Verification items for the finished model (mm, model axes). Face numbers are marked on the shaded views. A direction names the side the tool comes from. Round coordinates to 2 decimals unless told otherwise and drop trailing zeros. Write each loop counter-clockwise with the first axis right and the second up, starting at its lowest first coordinate (ties: lowest second). Pieces come first, ordered by that corner, then holes.
from build123d import *

# Parameters (mm, degrees)
FORMED_BRACKET_BODY_DEPTH = 150
BOSS_TUBE_SKETCH_R        = 112.5
BOSS_TUBE_SKETCH_R_2      = 87.5
BOSS_TUBE_225X170_DEPTH   = 170
BASE_HOLE_75_REACH        = 541.805
BASE_HOLE_SKETCH_R        = 37.5


with BuildPart() as part:
    # Bracket Profile Sketch → Formed Bracket Body (new, symmetric)
    with BuildSketch(Plane.XY):
        with BuildLine():
            Line((-475, 0), (-237.5, 0))
            ThreePointArc((-237.5, 0), (-202.144660941, -14.644660941), (-187.5, -50))
            Line((-187.5, -50), (-187.5, -188))
            ThreePointArc((-187.5, -188), (-181.642135624, -202.142135624), (-167.5, -208))
            Line((-167.5, -208), (167.5, -208))
            ThreePointArc((167.5, -208), (181.642135624, -202.142135624), (187.5, -188))
            Line((187.5, -188), (187.5, -50))
            ThreePointArc((187.5, -50), (202.144660941, -14.644660941), (237.5, 0))
            Line((237.5, 0), (475, 0))
            Line((475, 0), (475, -30))
            Line((475, -30), (237.5, -30))
            ThreePointArc((237.5, -30), (223.357864376, -35.857864376), (217.5, -50))
            Line((217.5, -50), (217.5, -188))
            ThreePointArc((217.5, -188), (202.855339059, -223.355339059), (167.5, -238))
            Line((167.5, -238), (-167.5, -238))
            ThreePointArc((-167.5, -238), (-202.855339059, -223.355339059), (-217.5, -188))
            Line((-217.5, -188), (-217.5, -50))
            ThreePointArc((-217.5, -50), (-223.357864376, -35.857864376), (-237.5, -30))
            Line((-237.5, -30), (-475, -30))
            Line((-475, -30), (-475, 0))
        make_face()
    extrude(amount=FORMED_BRACKET_BODY_DEPTH, both=True)

    # Boss Tube Sketch → Boss Tube Ø225x170 (add)
    with BuildSketch(Plane(origin=(0, -208, 0), x_dir=(1, 0, 0), z_dir=(0, 1, 0))):
        with Locations(Location((0, 0, 0), (0, 0, 180))):
            Circle(BOSS_TUBE_SKETCH_R)
        with Locations(Location((0, 0, 0), (0, 0, 180))):
            Circle(BOSS_TUBE_SKETCH_R_2, mode=Mode.SUBTRACT)
    extrude(amount=BOSS_TUBE_225X170_DEPTH)

    # Base Hole Sketch → Base Hole Ø75 (cut, up to next)
    with BuildSketch(Plane(origin=(0, -208, 0), x_dir=(1, 0, 0), z_dir=(0, 1, 0)), mode=Mode.PRIVATE) as base_hole_75_sk1:
        with Locations(Location((0, 0, 0), (0, 0, 180))):
            Circle(BASE_HOLE_SKETCH_R)
    base_hole_75_tool1 = extrude(base_hole_75_sk1.sketch, amount=-BASE_HOLE_75_REACH, mode=Mode.PRIVATE) & part.part
    add(base_hole_75_tool1.solids().sort_by_distance((0, -208, 0))[0], mode=Mode.SUBTRACT)


solid = part.part
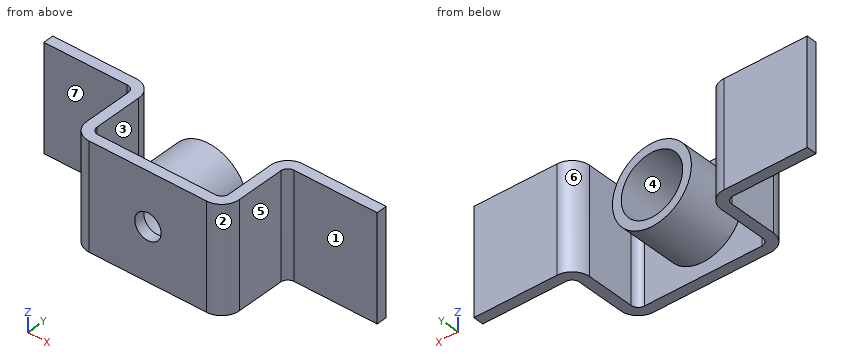
Q1. Depth check by flat-ended pin: P1, Ø12, axis at y = -172, z = -43.5, coming from the +X side; P2, Ø4, axis at y = -113, z = 65.5, coming from the -X side; P3, Ø8, axis at x = 103.5, y = -115, coming from the +Z side. Enter the tip coordinate at first touch or a pass-through.
Recorded:
P1: stops at x = 217.5
P2: stops at x = -217.5
P3: stops at z = 52.5
Q2. Release check for a two-part mould opening along X. For the marked faces 1, 2 and 3 record: released by +X, released by -X, zero draft, split by the parting line, or undercut.
Recorded:
face 1: zero draft
face 2: released by +X
face 3: undercut
Q3. Tool access check on the marked faces 4, 5, 6 and 7. Record the directions out of +Z, -Z, +X, -X, +Y, -Y that give a thin tool (end or side, any length) a straight path to the whole face; none if there is none.
Recorded:
face 4: +Y
face 5: +Z, -Z, +X, -Y
face 6: +Z, -Z, +Y
face 7: +Z, -Z, -X, -Y
Q4. Sectioned sample at D-D (x = 331). Enter the section's corners in (y, z).
Recorded:
outline: (-30, -150) - (0, -150) - (0, 150) - (-30, 150) - close
Q5. Material ranges on line 1 along Z through (x, y) = (0, -89); line 2 along X through (y, z) = (-158.5, -40); line 3 along X through (y, z) = (-141, 64.5), recorded low to high.
Recorded:
line 1: z = -112.5 to -87.5, 87.5 to 112.5
line 2: x = -217.5 to -187.5, -105.15 to -77.82, 77.82 to 105.15, 187.5 to 217.5
line 3: x = -217.5 to -187.5, -92.17 to -59.13, 59.13 to 92.17, 187.5 to 217.5
Q6. Sectioned sample at A-A (y = -164). Enter the section's corners in (x, z).
Recorded:
outline: (-217.5, -150) - (-187.5, -150) - (-187.5, 150) - (-217.5, 150) - close; circle Ø225 at (0, 0); (187.5, -150) - (217.5, -150) - (217.5, 150) - (187.5, 150) - close; hole circle Ø175 at (0, 0)
Q7. Sectioned sample at B-B (x = 0). Enter the section's corners in (y, z), plus the area to 4 significant figures.
Recorded:
outline: (-238, -150) - (-208, -150) - (-208, -112.5) - (-38, -112.5) - (-38, -87.5) - (-208, -87.5) - (-208, -37.5) - (-238, -37.5) - close; (-238, 37.5) - (-208, 37.5) - (-208, 87.5) - (-38, 87.5) - (-38, 112.5) - (-208, 112.5) - (-208, 150) - (-238, 150) - close
area: 15,250 mm2
